The listing builds one solid part. Answer for the finished solid, in the listing's coordinates (mm). A direction names the side the tool comes from. Coordinates: 2 decimals unless noted, no trailing zeros. Loops run counter-clockwise (first coordinate to the right, second up) from the corner with the lowest first, then second, coordinate; pieces in that order, holes last. Notation, with made-up numbers: (83, -12.5) - (103, -12.5) arc R24 ccw to (103, 23.5) - close; hole circle Ø5 at (71, 11.25). An arc over 180 degrees is marked (long way). Put each result on its own line as item: value.
```python
from build123d import *

# Parameters (mm, degrees)
BASE_PLATE_SKETCH_W                        = 75
BASE_PLATE_SKETCH_H                        = 45
BASE_PLATE_75X45X10_DEPTH                  = 10
LUG_PROFILE_SKETCH_W                       = 30
LUG_PROFILE_SKETCH_H                       = 10
CLEVIS_LUG_DEPTH                           = 35
LUG_TOP_CHAMFERS_5MM_SIZE                  = 5
BASE_PLATE_EDGE_CHAMFER_2MM_SIZE           = 2
MOUNTING_HOLE_SKETCH_R                     = 3.25
MOUNTING_HOLE_6_5_DEPTH                    = 57.013391256
MOUNTING_HOLES_MIRROR_RIGHT_COPY_1_SKETC_R = 3.25
MOUNTING_HOLES_MIRROR_RIGHT_COPY_1_DEPTH   = 57.013391256
PIN_BORE_SKETCH_R                          = 7.5
PIN_BORE_15_DEPTH                          = 70.552138716


with BuildPart() as part:
    # Base Plate Sketch → Base Plate 75x45x10 (new body)
    with BuildSketch(Plane(origin=(0, 0, 0), x_dir=(1, 0, 0), z_dir=(0, 1, 0))):
        Rectangle(BASE_PLATE_SKETCH_W, BASE_PLATE_SKETCH_H)
    extrude(amount=BASE_PLATE_75X45X10_DEPTH)

    # Lug Profile Sketch → Clevis Lug (add)
    with BuildSketch(Plane(origin=(0, 10, 0), x_dir=(1, 0, 0), z_dir=(0, 1, 0))):
        with Locations((0, -10)):
            Rectangle(LUG_PROFILE_SKETCH_W, LUG_PROFILE_SKETCH_H)
    clevis_lug = extrude(amount=CLEVIS_LUG_DEPTH)

    # Clevis Lug Mirror: Clevis Lug across plane
    add(clevis_lug.mirror(Plane.XY))

    # Lug Top Chamfers 5mm
    lug_top_chamfers_5mm_edges = [part.edges().sort_by_distance(p)[0] for p in [
        (15, 45, 10),
        (-15, 45, 10),
        (15, 45, -10),
        (-15, 45, -10),
    ]]
    chamfer(lug_top_chamfers_5mm_edges, length=LUG_TOP_CHAMFERS_5MM_SIZE)

    # Base Plate Edge Chamfer 2mm
    base_plate_edge_chamfer_2mm_edges = [part.edges().sort_by_distance(p)[0] for p in [
        (-37.5, 5, -22.5),
        (37.5, 5, -22.5),
        (37.5, 5, 22.5),
        (-37.5, 5, 22.5),
    ]]
    chamfer(base_plate_edge_chamfer_2mm_edges, length=BASE_PLATE_EDGE_CHAMFER_2MM_SIZE)

    # Mounting Hole Sketch → Mounting Hole Ø6.5 (cut, through all)
    with BuildSketch(Plane(origin=(0, 10, 0), x_dir=(1, 0, 0), z_dir=(0, 1, 0))):
        with Locations(Location((-30.5, 15.5, 0), (0, 0, 270))):
            Circle(MOUNTING_HOLE_SKETCH_R)
    mounting_hole_6_5 = extrude(amount=-MOUNTING_HOLE_6_5_DEPTH, mode=Mode.SUBTRACT)

    # Mounting Hole Mirror Front: Mounting Hole Ø6.5 across plane
    add(mounting_hole_6_5.mirror(Plane.XY), mode=Mode.SUBTRACT)

    # Mounting Holes Mirror Right: Mounting Hole Ø6.5 across plane
    add(mounting_hole_6_5.mirror(Plane(origin=(0, 0, 0), x_dir=(0, 0, 1), z_dir=(1, 0, 0))), mode=Mode.SUBTRACT)

    # Mounting Holes Mirror Right copy 1 sketc → Mounting Holes Mirror Right copy 1 (cut, through all)
    with BuildSketch(Plane(origin=(0, 10, 0), x_dir=(-1, 0, 0), z_dir=(0, 1, 0))):
        with Locations(Location((-30.5, 15.5, 0), (0, 0, 270))):
            Circle(MOUNTING_HOLES_MIRROR_RIGHT_COPY_1_SKETC_R)
    extrude(amount=-MOUNTING_HOLES_MIRROR_RIGHT_COPY_1_DEPTH, mode=Mode.SUBTRACT)

    # Pin Bore Sketch → Pin Bore Ø15 (cut, through all)
    with BuildSketch(Plane.XY.offset(15)):
        with Locations((0, 30)):
            Circle(PIN_BORE_SKETCH_R)
    extrude(amount=-PIN_BORE_15_DEPTH, mode=Mode.SUBTRACT)


solid = part.part
```
1) The part is cut by section A-A (x = 0). Give the vertices of the cut face in (y, z), and give its area (3 significant figures).
Found:
outline: (0, -22.5) - (10, -22.5) - (10, -15) - (22.5, -15) - (22.5, -5) - (10, -5) - (10, 5) - (22.5, 5) - (22.5, 15) - (10, 15) - (10, 22.5) - (0, 22.5) - close; (37.5, -15) - (45, -15) - (45, -5) - (37.5, -5) - close; (37.5, 5) - (45, 5) - (45, 15) - (37.5, 15) - close
area: 850 mm^2
2) Straight lines are drawn through the part: L1, parallel to X at y = 7.25, z = 15.5; L2, parallel to Y at x = 0, z = 9.5; L3, parallel to Z at x = 30.5, y = 2. For each, find the intervals that lie inside material, in ascending order. Write a range as [from, to].
Found:
L1: x = [-37.5, -33.75], [-27.25, 27.25], [33.75, 37.5]
L2: y = [0, 22.5], [37.5, 45]
L3: z = [-22.5, -18.75], [-12.25, 12.25], [18.75, 22.5]
3) The part is cut by section B-B (y = 3). Give the vertices of the cut face in (x, z).
Found:
outline: (-37.5, -20.5) - (-35.5, -22.5) - (35.5, -22.5) - (37.5, -20.5) - (37.5, 20.5) - (35.5, 22.5) - (-35.5, 22.5) - (-37.5, 20.5) - close; hole circle Ø6.5 at (-30.5, -15.5); hole circle Ø6.5 at (-30.5, 15.5); hole circle Ø6.5 at (30.5, -15.5); hole circle Ø6.5 at (30.5, 15.5)
4) Each of these flat-tipped pins is pushed along its axis until it touches: pin 1 (24 mm diameter, centred on x = -1, y = 33.5, fed in from +Z); pin 2 (3 mm diameter, centred on y = 28.5, z = 12, fed in from +X); pin 3 (5 mm diameter, centred on y = 20, z = 15.5, fed in from -X). Where does it stop, or does it pass through?
Found:
pin 1: stops at z = 15
pin 2: stops at x = 15
pin 3: stops at x = -15
5) The part is cut by section D-D (y = 41). Give the vertices of the cut face in (x, z), and give its area (3 significant figures).
Found:
outline: (-14, -15) - (14, -15) - (14, -5) - (-14, -5) - close; (-14, 5) - (14, 5) - (14, 15) - (-14, 15) - close
area: 560 mm^2
6) For faces 4 (the face through (-1, 10, 0)), 5 (the face through (-15, 25, 10)), 6 (the face through (15, 25, 10)), determine the directions among +Z, -Z, +X, -X, +Y, -Y from which every point of the face is accessible in a straight line to the end or side of a thin tool.
Found:
face 4: +Y
face 5: +Z, -Z, -X, +Y
face 6: +Z, -Z, +X, +Y
7) For a pull along Z with two mould halves and no side action, classify faces 1 (the face through (0, 5, -22.5)), 2 (the face through (-12, 43, 10)), 3 (the face through (-33.673, 5.07, -16.205)) as pulls with the +Z half, pulls with the -Z half, needs draft (parallel to the pull), parting line crosses it, or undercut.
Found:
face 1: pulls with the -Z half
face 2: needs draft
face 3: undercut
8) The part is cut by section C-C (z = -9.5). Give the vertices of the cut face in (x, y), and give its area (3 significant figures).
Found:
outline: (-37.5, 0) - (37.5, 0) - (37.5, 10) - (15, 10) - (15, 40) - (10, 45) - (-10, 45) - (-15, 40) - (-15, 10) - (-37.5, 10) - close; hole circle Ø15 at (0, 30)
area: 1,600 mm^2
